Verification items for the finished model (mm, model axes). Face numbers are marked on the shaded views. A direction names the side the tool comes from. Coordinates: 2 decimals unless noted, no trailing zeros. Loops run counter-clockwise (first coordinate to the right, second up) from the corner with the lowest first, then second, coordinate; pieces in that order, holes last.
Q1. Mould release check, pull along X, two halves, no side actions. Record for the marked faces 1, 2 and 3: +X half, -X half, draft (parallel to the pull), parting line (faces both ways), or undercut.
Q2. Sectioned sample at C-C (z = 125). Enter the section's corners in (x, y).
Q3. Go/stop test with a flat-tipped pin: P1, Ø3, axis at x = 20.5, z = 57, coming from the -Y side. Record where the tip stops, or that it passes through.
Q4. Material ranges on probe 1 along Y at (x, z) = (22.5, 76), recorded low to high.
Q5. Access from +Z, -Z, +X, -X, +Y, -Y to the whole of each face (thin tool, end or side, straight path). Record for the marked faces 4 and 5.
Q6. Sectioned sample at A-A (x = 25.25). Enter the section's corners in (y, z), then the cut area to 3 significant figures.
```python
from build123d import *

# Parameters (mm, degrees)
SKETCH_1_W          = 30
SKETCH_1_H          = 30
SKETCH_1_W_2        = 24
SKETCH_1_H_2        = 24
EXTRUDE_1_DEPTH     = 150
SKETCH_2_W          = 30
SKETCH_2_H          = 30
CUT_EXTRUDE_1_DEPTH = 40


with BuildPart() as part:
    # 草图1 → 凸台-拉伸1 (new body)
    with BuildSketch(Plane.XY):
        with Locations((15, 15)):
            Rectangle(SKETCH_1_W, SKETCH_1_H)
        with Locations((15, 15)):
            Rectangle(SKETCH_1_W_2, SKETCH_1_H_2, mode=Mode.SUBTRACT)
    extrude(amount=EXTRUDE_1_DEPTH)

    # 草图2 → 切除-拉伸1 (cut)
    with BuildSketch(Plane(origin=(0, 0, 0), x_dir=(-1, 0, 0), z_dir=(0, 0, -1))):
        with Locations((-15, 15)):
            Rectangle(SKETCH_2_W, SKETCH_2_H)
    extrude(amount=-CUT_EXTRUDE_1_DEPTH, mode=Mode.SUBTRACT)


solid = part.part
```
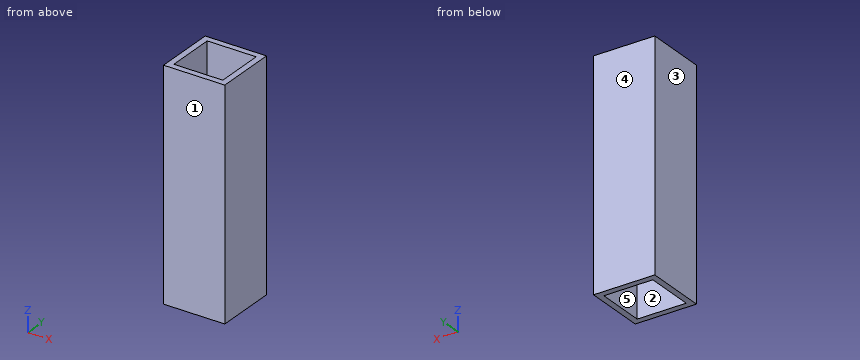
Geometry check:
1. face 1: draft
1. face 2: undercut
1. face 3: -X half
2. outline: (0, 0) - (30, 0) - (30, 30) - (0, 30) - close; hole (3, 3) - (27, 3) - (27, 27) - (3, 27) - close
3. P1: stops at y = 0
4. probe 1: y = 0 to 3, 27 to 30
5. face 4: +Z, -Z, +X, -X, +Y
5. face 5: +Z, -Z
6. outline: (0, 40) - (3, 40) - (3, 150) - (0, 150) - close; (27, 40) - (30, 40) - (30, 150) - (27, 150) - close
6. area: 660 mm2
